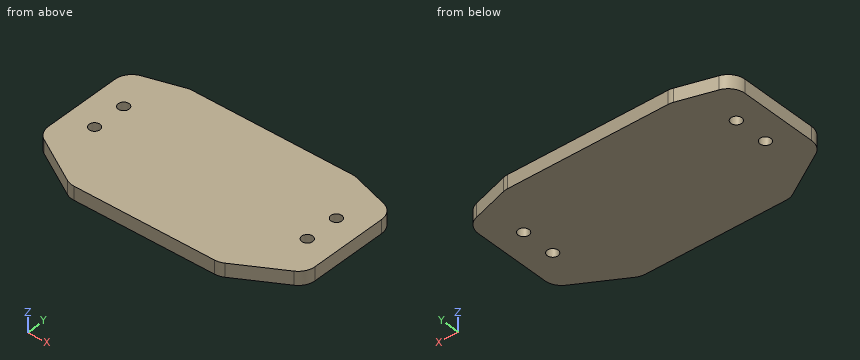
```python
from build123d import *

# Parameters (mm, degrees)
SKETCH_1_R      = 1.6
EXTRUDE_1_DEPTH = 4
FILLET_R5_1_R   = 5


with BuildPart() as part:
    # 草图1 → 凸台-拉伸1 (new body)
    with BuildSketch(Plane.XY):
        Polygon((-24.5, 23.5), (24.5, 23.5), (39.5, 19), (39.5, -10.5), (22.179491924, -20.5), (-22.179491924, -20.5), (-39.5, -10.5), (-39.5, 19), align=None)
        with Locations((-31.5, 9)):
            Circle(SKETCH_1_R, mode=Mode.SUBTRACT)
        with Locations((-31.5, -1)):
            Circle(SKETCH_1_R, mode=Mode.SUBTRACT)
        with Locations(Location((31.5, -1, 0), (0, 0, 180))):
            Circle(SKETCH_1_R, mode=Mode.SUBTRACT)
        with Locations(Location((31.5, 9, 0), (0, 0, 180))):
            Circle(SKETCH_1_R, mode=Mode.SUBTRACT)
    extrude(amount=EXTRUDE_1_DEPTH)

    # R5 圆角1
    fillet_r5_1_edges = [part.edges().sort_by_distance(p)[0] for p in [
        (-24.5, 23.5, 2),
        (24.5, 23.5, 2),
        (39.5, 19, 2),
        (39.5, -10.5, 2),
        (22.179491924, -20.5, 2),
        (-22.179491924, -20.5, 2),
        (-39.5, -10.5, 2),
        (-39.5, 19, 2),
    ]]
    fillet(fillet_r5_1_edges, radius=FILLET_R5_1_R)


solid = part.part
```
Here's how the part is built. I have some questions about the finished solid (model axes, mm). Coordinates: 2 decimals unless noted, no trailing zeros. Order: outer loops, then holes, each group sorted by start corner. A loop starts at its lowest first (then second) coordinate and runs counter-clockwise, first axis right, second up.
1) Imagine slicing it at A-A on y = 9. List the corners of the cut face in (x, z) for me.
2) Imagine slicing it at C-C on z = 2.05. List the corners of the cut face in (x, y) for me, and give its area (3 significant figures).
3) Imagine slicing it at D-D on y = -14.5. List the corners of the cut face in (x, z) for me.
4) I need wall thicknesses on line 1 (Y direction, x = 31.5, z = 2.45); line 2 (Y direction, x = 32, z = 3.25); line 3 (Y direction, x = -24, z = 1.85). Which ranges of each line are inside material? Lowest first, please.
5) Imagine slicing it at B-B on x = -31.5. List the corners of the cut face in (y, z) for me, and give its area (3 significant figures).
6) Will this pin go through, and if not, where does the flat tip stop? pin 1 (4 mm diameter, centred on x = -31.5, y = 9, fed in from +Z).
Response values:
1. outline: (-39.5, 0) - (-33.1, 0) - (-33.1, 4) - (-39.5, 4) - close; (-29.9, 0) - (29.9, 0) - (29.9, 4) - (-29.9, 4) - close; (33.1, 0) - (39.5, 0) - (39.5, 4) - (33.1, 4) - close
2. outline: (-39.5, -7.61) arc R5 ccw to (-37, -11.94) - (-23.34, -19.83) arc R5 ccw to (-20.84, -20.5) - (20.84, -20.5) arc R5 ccw to (23.34, -19.83) - (37, -11.94) arc R5 ccw to (39.5, -7.61) - (39.5, 15.28) arc R5 ccw to (35.94, 20.07) - (25.2, 23.29) arc R5 ccw to (23.77, 23.5) - (-23.77, 23.5) arc R5 ccw to (-25.2, 23.29) - (-35.94, 20.07) arc R5 ccw to (-39.5, 15.28) - close; hole circle Ø3.2 at (-31.5, -1); hole circle Ø3.2 at (-31.5, 9); hole circle Ø3.2 at (31.5, -1); hole circle Ø3.2 at (31.5, 9)
2. area: 3,190 mm2
3. outline: (-32.57, 0) - (32.57, 0) - (32.57, 4) - (-32.57, 4) - close
4. line 1: y = -15.12 to -2.6, 0.6 to 7.4, 10.6 to 21.4
4. line 2: y = -14.83 to -2.52, 0.52 to 7.48, 10.52 to 21.25
4. line 3: y = -19.45 to 23.49
5. outline: (-15.12, 0) - (-2.6, 0) - (-2.6, 4) - (-15.12, 4) - close; (0.6, 0) - (7.4, 0) - (7.4, 4) - (0.6, 4) - close; (10.6, 0) - (21.4, 0) - (21.4, 4) - (10.6, 4) - close
5. area: 120 mm2
6. pin 1: stops at z = 4
